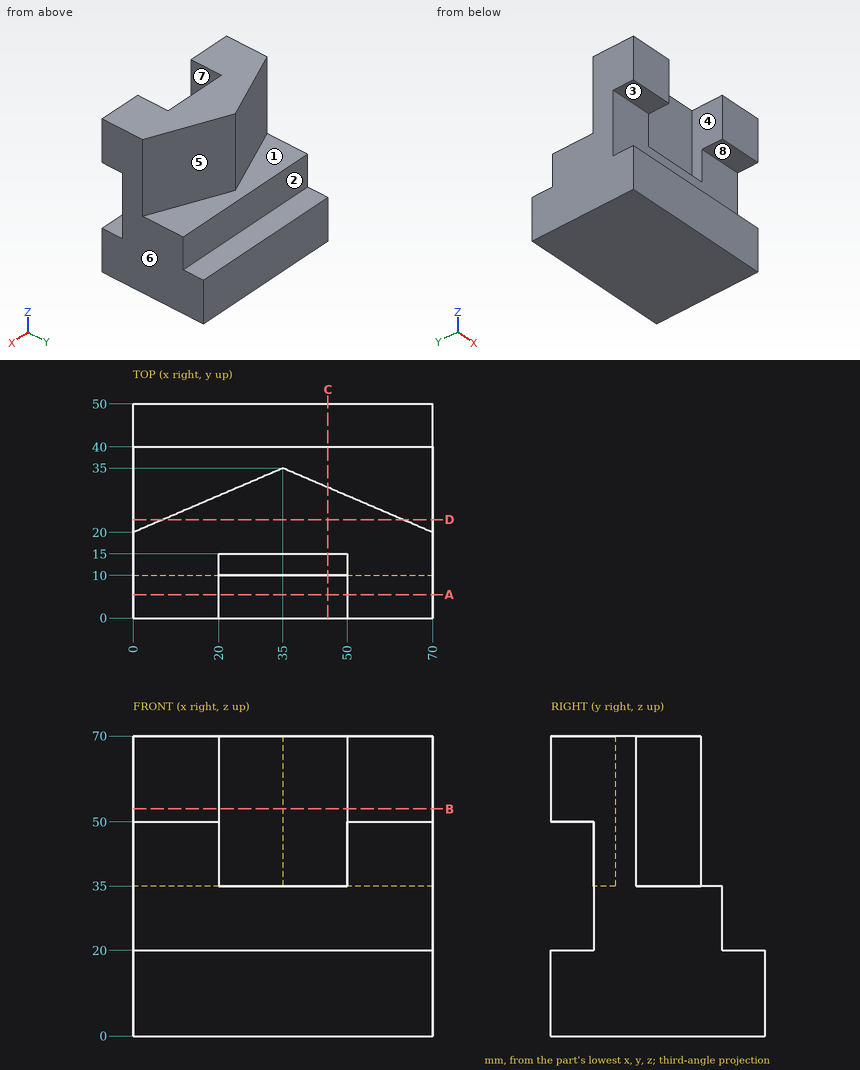
Can you work these out from the drawing? Everything is in mm from the part's minimum corner. A direction names the side the tool comes from. Coordinates: 2 decimals unless noted, no trailing zeros. Loops run counter-clockwise (first coordinate to the right, second up) from the corner with the lowest first, then second, coordinate; pieces in that order, holes last. Notation, with made-up numbers: (14.5, 1) - (20.5, 1) arc R22 cw to (20.5, 20) - close; hole circle Ø4 at (-11.75, 89.5). An arc over 180 degrees is marked (long way). Use a Markdown table: item, result.
Item 1: I want a section at A-A on y = 5.5. Please give me the cut outline in (x, z), and give its area (3 significant figures).
Numbers:
| item | result |
|---|---|
| outline | (0, 0) - (70, 0) - (70, 20) - (0, 20) - close; (0, 50) - (20, 50) - (20, 70) - (0, 70) - close; (50, 50) - (70, 50) - (70, 70) - (50, 70) - close |
| area | 2,200 mm2 |
Item 2: If I drill on probe 1 along Z at (x, y) = (11.5, 8); probe 2 along Z at (x, y) = (3, 29.5), over which ranges is the centre line in solid material (lowest first)? Write a range as from..to.
Numbers:
| item | result |
|---|---|
| probe 1 | z = 0..20, 50..70 |
| probe 2 | z = 0..35 |
Item 3: We'd pull the mould along X, two halves only. Please class the marked faces 6, 7 and 8: released by +X, released by -X, zero draft, split by the parting line, or undercut.
Numbers:
| item | result |
|---|---|
| face 6 | released by +X |
| face 7 | undercut |
| face 8 | zero draft |
Item 4: Will these pins go through, and if not, where does the flat tip stop? pin 1 (1 mm diameter, centred on y = 35, z = 62.5, fed in from -X); pin 2 (24 mm diameter, centred on x = 33.5, z = 57, fed in from -Y); pin 3 (5 mm diameter, centred on x = 30.5, z = 58, fed in from +Y); pin 4 (4.5 mm diameter, centred on y = 7, z = 46.5, fed in from +X).
Numbers:
| item | result |
|---|---|
| pin 1 | stops at x = 33.83 |
| pin 2 | stops at y = 15 |
| pin 3 | stops at y = 34.14 |
| pin 4 | passes through |
Item 5: I want a section at B-B on z = 53. Please give me the cut outline in (x, y), and give its area (4 significant figures).
Numbers:
| item | result |
|---|---|
| outline | (0, 0) - (20, 0) - (20, 15) - (50, 15) - (50, 0) - (70, 0) - (70, 20) - (35, 35) - (0, 20) - close |
| area | 1,475 mm2 |
Item 6: I want a section at D-D on y = 23. Please give me the cut outline in (x, z).
Numbers:
| item | result |
|---|---|
| outline | (0, 0) - (70, 0) - (70, 35) - (63, 35) - (63, 70) - (7, 70) - (7, 35) - (0, 35) - close |
Item 7: For the marked faces 1, 2, 3, 4 and 5, which set-ups out of +Z, -Z, +X, -X, +Y, -Y let a thin tool reach every point of the face, with its end or its side?
Numbers:
| item | result |
|---|---|
| face 1 | +Z, +Y |
| face 2 | +Z, +X, -X, +Y |
| face 3 | +X, -X, -Y |
| face 4 | +Z, -Y |
| face 5 | +Z, +X, +Y |
Item 8: I want a section at C-C on x = 45.5. Please give me the cut outline in (y, z).
Numbers:
| item | result |
|---|---|
| outline | (0, 0) - (50, 0) - (50, 20) - (40, 20) - (40, 35) - (30.5, 35) - (30.5, 70) - (15, 70) - (15, 35) - (10, 35) - (10, 20) - (0, 20) - close |
